Here's how the part is built. I have some questions about the finished solid (model axes, mm). Round coordinates to 2 decimals unless told otherwise and drop trailing zeros. Order: outer loops, then holes, each group sorted by start corner. A loop starts at its lowest first (then second) coordinate and runs counter-clockwise, first axis right, second up.
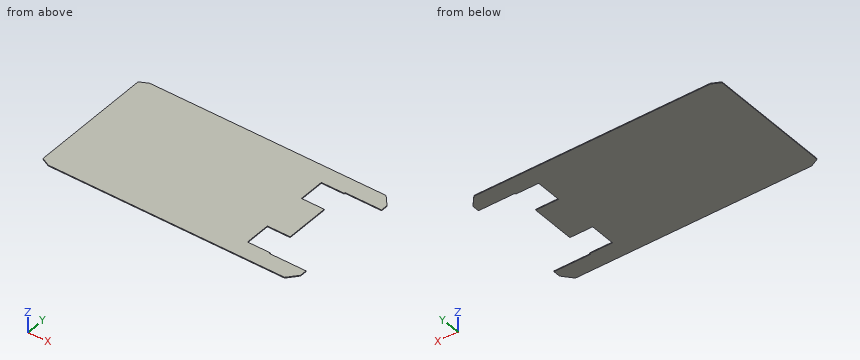
```python
from build123d import *

# Parameters (mm, degrees)
EXTRUDE_1_DEPTH     = 1.5
SKETCH_2_W          = 102
SKETCH_2_H          = 92
CUT_EXTRUDE_1_DEPTH = 15


with BuildPart() as part:
    # 草图1 → 凸台-拉伸1 (new, symmetric)
    with BuildSketch(Plane.XY):
        Polygon((-620, -220), (-590, -235), (250, -235), (280, -200), (280, -175), (150, -175), (150, 175), (280, 175), (280, 200), (250, 235), (-590, 235), (-620, 220), align=None)
    extrude(amount=EXTRUDE_1_DEPTH, both=True)

    # 草图2 → 切除-拉伸1 (cut, symmetric)
    with BuildSketch(Plane.XY):
        with Locations((120, 125)):
            Rectangle(SKETCH_2_W, SKETCH_2_H)
        with Locations((120, -125)):
            Rectangle(SKETCH_2_W, SKETCH_2_H)
    extrude(amount=CUT_EXTRUDE_1_DEPTH, both=True, mode=Mode.SUBTRACT)


solid = part.part
```
1. I need wall thicknesses on probe 1 along Y at (x, z) = (125, -0.75); probe 2 along Y at (x, z) = (222, 0.6); probe 3 along X at (y, z) = (63.5, -0.55). Which ranges of each line are inside material? Lowest first, please.
Evaluation:
probe 1: y = -235 to -171, -79 to 79, 171 to 235
probe 2: y = -235 to -175, 175 to 235
probe 3: x = -620 to 150
2. If we section it at D-D, the plane y = 161.5: Write out the boundary of the cut face in (x, z), and give its area (3 significant figures).
Evaluation:
outline: (-620, -1.5) - (69, -1.5) - (69, 1.5) - (-620, 1.5) - close
area: 2,070 mm2
3. I'm going to push a flat-ended pin straight in: P1, Ø0.9, axis at y = -135.5, z = -0.5, coming from the +X side. Where does the tip first touch, or does it pass through?
Evaluation:
P1: stops at x = 69
4. If we section it at C-C, the plane y = 11: Write out the boundary of the cut face in (x, z).
Evaluation:
outline: (-620, -1.5) - (150, -1.5) - (150, 1.5) - (-620, 1.5) - close
5. If we section it at A-A, the plane x = 204: Write out the boundary of the cut face in (y, z).
Evaluation:
outline: (-235, -1.5) - (-175, -1.5) - (-175, 1.5) - (-235, 1.5) - close; (175, -1.5) - (235, -1.5) - (235, 1.5) - (175, 1.5) - close
6. If we section it at B-B, the plane z = -0.5: Write out the boundary of the cut face in (x, y).
Evaluation:
outline: (-620, -220) - (-590, -235) - (250, -235) - (280, -200) - (280, -175) - (150, -175) - (150, -171) - (69, -171) - (69, -79) - (150, -79) - (150, 79) - (69, 79) - (69, 171) - (150, 171) - (150, 175) - (280, 175) - (280, 200) - (250, 235) - (-590, 235) - (-620, 220) - close
